from build123d import *

# Parameters (mm, degrees)
CHAMFER_1_SIZE      = 0.5
CUT_EXTRUDE_START   = -11
CUT_EXTRUDE_1_DEPTH = 10
SKETCH_11_R         = 20.368798622
SKETCH_11_R_2       = 14.3
CUT_EXTRUDE_3_DEPTH = 1.75
CHAMFER_3_SIZE      = 0.5


with BuildPart() as part:
    # 草图1 → 旋转1 (revolve)
    with BuildSketch(Plane(origin=(0, 0, 0), x_dir=(-1, 0, 0), z_dir=(0, 0, -1)), mode=Mode.PRIVATE) as revolve_1_sk:
        Polygon((-60, 17.5), (60, 17.5), (60, 15), (93, 15), (93, 12.5), (138, 12.5), (138, 0), (-138, 0), (-138, 12.5), (-93, 12.5), (-93, 15), (-60, 15), align=None)
    revolve(revolve_1_sk.sketch.rotate(Axis((70, 0, 0), (-1, 0, 0)), 270), axis=Axis((70, 0, 0), (-1, 0, 0)))

    # 倒角1
    chamfer_1_edges = [part.edges().sort_by_distance(p)[0] for p in [
        (-138, 0, -12.5),
        (-93, 0, -15),
        (-60, 0, -17.5),
        (60, 0, -17.5),
        (93, 0, -15),
    ]]
    chamfer(chamfer_1_edges, length=CHAMFER_1_SIZE)

    # 草图2 → 切除-拉伸1 (cut)
    with BuildSketch(Plane.XY.offset(CUT_EXTRUDE_START)):
        with BuildLine():
            Line((-77, 4), (-65, 4))
            ThreePointArc((-65, 4), (-61, 0), (-65, -4))
            Line((-65, -4), (-77, -4))
            ThreePointArc((-77, -4), (-81, 0), (-77, 4))
        make_face()
        with BuildLine():
            Line((65, 4), (77, 4))
            ThreePointArc((77, 4), (81, 0), (77, -4))
            Line((77, -4), (65, -4))
            ThreePointArc((65, -4), (61, 0), (65, 4))
        make_face()
    extrude(amount=-CUT_EXTRUDE_1_DEPTH, mode=Mode.SUBTRACT)

    # 草图11 → 切除-拉伸3 (cut)
    with BuildSketch(Plane(origin=(82, 0, 0), x_dir=(0, 0, -1), z_dir=(1, 0, 0))):
        Circle(SKETCH_11_R)
        Circle(SKETCH_11_R_2, mode=Mode.SUBTRACT)
    cut_extrude_3 = extrude(amount=CUT_EXTRUDE_3_DEPTH, mode=Mode.SUBTRACT)

    # 镜向1: 切除-拉伸3 across plane
    add(cut_extrude_3.mirror(Plane(origin=(0, 0, 0), x_dir=(0, 0, 1), z_dir=(1, 0, 0))), mode=Mode.SUBTRACT)

    # 倒角3
    chamfer_3_edges = [part.edges().sort_by_distance(p)[0] for p in [
        (138, 0, -12.5),
    ]]
    chamfer(chamfer_3_edges, length=CHAMFER_3_SIZE)


solid = part.part
Here's how the part is built. I have some questions about the finished solid (model axes, mm). A direction names the side the tool comes from. Coordinates: 2 decimals unless noted, no trailing zeros. Write each loop counter-clockwise with the first axis right and the second up, starting at its lowest first coordinate (ties: lowest second). Pieces come first, ordered by that corner, then holes. Notation, with made-up numbers: (-37.5, -6) - (-32.5, -6) arc R26 cw to (-32.5, 27) - close; hole circle Ø8 at (-9.75, 80). An arc over 180 degrees is marked (long way). Use one line per item in the form item = value.
1) Thinking about a two-plate mould opening in X: for faces 5 (the flat face through (-93, 7, -11)), 6 (the flat face through (71, 0, -11)), 7 (the flat face through (-71, 0, -11)), 8 (the cylindrical face through (114.938, 3.755, 11.923)), which applies, released by +X, released by -X, zero draft, split by the parting line, or undercut?
Solved:
face_5 = released by -X
face_6 = undercut
face_7 = undercut
face_8 = zero draft
2) On a 3-axis mill with a long thin cutter (end or side, diameter ignored), from which of +Z, -Z, +X, -X, +Y, -Y can I reach the whole of each face in a straight line? I mean faces 1 (the cylindrical face through (-82.86, 14.18, 1.86)), 2 (the flat face through (60, -14, -6)), 3 (the cylindrical face through (-71.154, -5.745, 13.856)), 4 (the cylindrical face through (-0.833, -10.648, -13.887)). Say none if no direction works.
Solved:
face_1 = none
face_2 = +X
face_3 = -X
face_4 = +X, -X
3) I need wall thicknesses on line 1 (X direction, y = -0.5, z = -13); line 2 (Y direction, x = -92, z = -1); line 3 (Z direction, x = 25.5, y = 1). Which ranges of each line are inside material? Lowest first, please.
Solved:
line_1 = -93 to -80.97, -61.03 to 61.03, 80.97 to 93
line_2 = -14.97 to 14.97
line_3 = -17.47 to 17.47
4) Suppose I cut it at A-A, the plane x = -87.5. Write out the boundary of the cut face in (y, z).
Solved:
outline = circle Ø30 at (0, 0)
5) I'm going to push flat-ended pins straight in: P1, Ø1, axis at x = -70, z = -13.5, coming from the +Y side; P2, Ø1, axis at y = 12, z = -1, coming from the -X side; P3, Ø1, axis at x = -74, z = -12, coming from the -Y side; P4, Ø2, axis at x = 101.5, y = 8.5, coming from the +Z side. Where does each tip first touch, or does it pass through?
Solved:
P1 = 7.48
P2 = -138
P3 = -9.63
P4 = 10
6) Suppose I cut it at B-B, the plane x = 46. Write out the boundary of the cut face in (y, z).
Solved:
outline = circle Ø35 at (0, 0)
